```python
from build123d import *

# Parameters (mm, degrees)
CUT_EXTRUDE_1_DEPTH      = 205.5
CUT_EXTRUDE_1_DEPTH_BACK = 205.5
SKETCH_2_R               = 40
SKETCH_3_OUTSIDE_W       = 124.974
SKETCH_3_OUTSIDE_H       = 124.974
SKETCH_3_OUTSIDE_R       = 17.5
CUT_EXTRUDE_2_DEPTH      = 18
SKETCH_4_OUTSIDE_W       = 124.974
SKETCH_4_OUTSIDE_H       = 124.974
SKETCH_4_OUTSIDE_R       = 12.5
CUT_EXTRUDE_3_DEPTH      = 26
SKETCH_5_OUTSIDE_W       = 124.974
SKETCH_5_OUTSIDE_H       = 124.974
SKETCH_5_OUTSIDE_R       = 17.5
CUT_EXTRUDE_4_DEPTH      = 30
CUT_EXTRUDE_5_DEPTH      = 4
SKETCH_7_R               = 17.5
EXTRUDE_1_DEPTH          = 51
SKETCH_9_OUTSIDE_W       = 135.09
SKETCH_9_OUTSIDE_H       = 135.09
SKETCH_9_OUTSIDE_R       = 12
CUT_EXTRUDE_7_DEPTH      = 26
MOVE_FACE_1_BY           = 8


with BuildPart() as part:
    # 草图1 → 旋转1 (revolve)
    with BuildSketch(Plane.XY, mode=Mode.PRIVATE) as revolve_1_sk:
        Polygon((-205.5, 0), (-205.5, 19), (-204.5, 20), (204.5, 20), (205.5, 19), (205.5, 0), align=None)
    revolve(revolve_1_sk.sketch.rotate(Axis((205.5, 0, 0), (-1, 0, 0)), 270), axis=Axis((205.5, 0, 0), (-1, 0, 0)))

    # 草图2 → 切除-拉伸1 (cut, two sides: drawn at the far end of the back side and taken through both)
    with BuildSketch(Plane(origin=(0, 0, 0), x_dir=(0, 0, -1), z_dir=(1, 0, 0)).offset(-CUT_EXTRUDE_1_DEPTH_BACK)):
        Circle(SKETCH_2_R)
        with BuildLine():
            ThreePointArc((-19.926297295, 1.715423015), (-14.142135624, -14.142135624), (1.715423015, -19.926297295))
            ThreePointArc((1.715423015, -19.926297295), (3.302788339, -18.731043462), (5.203224708, -19.311303753))
            ThreePointArc((5.203224708, -19.311303753), (14.142135624, -14.142135624), (19.311303753, -5.203224708))
            ThreePointArc((19.311303753, -5.203224708), (18.731043462, -3.302788339), (19.926297295, -1.715423015))
            ThreePointArc((19.926297295, -1.715423015), (14.142135624, 14.142135624), (-1.715423015, 19.926297295))
            ThreePointArc((-1.715423015, 19.926297295), (-3.302788339, 18.731043462), (-5.203224708, 19.311303753))
            ThreePointArc((-5.203224708, 19.311303753), (-14.142135624, 14.142135624), (-19.311303753, 5.203224708))
            ThreePointArc((-19.311303753, 5.203224708), (-18.731043462, 3.302788339), (-19.926297295, 1.715423015))
        make_face(mode=Mode.SUBTRACT)
    extrude(amount=CUT_EXTRUDE_1_DEPTH + CUT_EXTRUDE_1_DEPTH_BACK, mode=Mode.SUBTRACT)

    # 草图3 outside → 切除-拉伸2 (cut)
    with BuildSketch(Plane.ZY.offset(205.5)):
        Rectangle(SKETCH_3_OUTSIDE_W, SKETCH_3_OUTSIDE_H)
        Circle(SKETCH_3_OUTSIDE_R, mode=Mode.SUBTRACT)
    extrude(amount=-CUT_EXTRUDE_2_DEPTH, mode=Mode.SUBTRACT)

    # 草图4 outside → 切除-拉伸3 (cut)
    with BuildSketch(Plane(origin=(205.5, 0, 0), x_dir=(0, 0, -1), z_dir=(1, 0, 0))):
        Rectangle(SKETCH_4_OUTSIDE_W, SKETCH_4_OUTSIDE_H)
        Circle(SKETCH_4_OUTSIDE_R, mode=Mode.SUBTRACT)
    extrude(amount=-CUT_EXTRUDE_3_DEPTH, mode=Mode.SUBTRACT)

    # 草图5 outside → 切除-拉伸4 (cut)
    with BuildSketch(Plane(origin=(179.5, 0, 0), x_dir=(0, 0, -1), z_dir=(1, 0, 0))):
        Rectangle(SKETCH_5_OUTSIDE_W, SKETCH_5_OUTSIDE_H)
        with Locations(Location((0, 0, 0), (0, 0, 180))):
            Circle(SKETCH_5_OUTSIDE_R, mode=Mode.SUBTRACT)
    extrude(amount=-CUT_EXTRUDE_4_DEPTH, mode=Mode.SUBTRACT)

    # 草图6 → 切除-拉伸5 (cut)
    with BuildSketch(Plane(origin=(0, 12.5, 0), x_dir=(1, 0, 0), z_dir=(0, 1, 0))):
        with BuildLine():
            Line((200.5, -4), (185.5, -4))
            ThreePointArc((185.5, -4), (181.5, 0), (185.5, 4))
            Line((185.5, 4), (200.5, 4))
            ThreePointArc((200.5, 4), (204.5, 0), (200.5, -4))
        make_face()
    cut_extrude_5 = extrude(amount=-CUT_EXTRUDE_5_DEPTH, mode=Mode.SUBTRACT)

    # 草图7 → 凸台-拉伸1 (add)
    with BuildSketch(Plane.ZY.offset(205.5)):
        Circle(SKETCH_7_R)
    extrude(amount=EXTRUDE_1_DEPTH)

    # 草图9 outside → 切除-拉伸7 (cut)
    with BuildSketch(Plane.ZY.offset(256.5)):
        Rectangle(SKETCH_9_OUTSIDE_W, SKETCH_9_OUTSIDE_H)
        Circle(SKETCH_9_OUTSIDE_R, mode=Mode.SUBTRACT)
    extrude(amount=-CUT_EXTRUDE_7_DEPTH, mode=Mode.SUBTRACT)

    # 镜向1: 切除-拉伸5 across plane
    add(cut_extrude_5.mirror(Plane.ZY.offset(25.5)), mode=Mode.SUBTRACT)

    # Move Face 1: a face moved outward by 8.0
    extrude(part.faces().sort_by_distance((-187.5, -16, -10))[0], amount=MOVE_FACE_1_BY, dir=(-1, 0, 0))


solid = part.part
```
Work out the finished part from the listing and answer in its coordinate system (mm). A direction names the side the tool comes from. Give positions to 0.01 mm unless a question says otherwise; leave off trailing zeros. Write each loop counter-clockwise with the first axis right and the second up, starting at its lowest first coordinate (ties: lowest second). Pieces come first, ordered by that corner, then holes. Notation, with made-up numbers: (3, 83.25) -> (18, 83.25) arc R9 ccw to (18, 89.25) -> close; hole circle Ø10 at (-35.5, 43.25). An arc over 180 degrees is marked (long way). Write each question's results on one line, items separated by ' | '.
1. A tool of negligible diameter and unlimited length cuts with its end or side. For faces 5 (the flat face through (-256.5, 0, 0)), 6 (the flat face through (193, 8.5, 0)), 7 (the cylindrical face through (-243.682, -11.715, -2.601)), 8 (the cylindrical face through (192.68, -11.09, -5.77)), from which of +Z, -Z, +X, -X, +Y, -Y can it reach the whole face along a straight path? Write none if from no direction.
Data:
face 5: +Z, -Z, -X, +Y, -Y | face 6: +Y | face 7: -X | face 8: +X
2. Straight lines are drawn through the part: L1, parallel to Y at x = -178.5, z = 5.5; L2, parallel to X at y = 11.5, z = -12; L3, parallel to Y at x = -94, z = 7 (3 decimals). For each, find the intervals that lie inside material, in ascending order.
Data:
L1: -19.23 to 19.23 | L2: -230.5 to 179.5 | L3: -18.735 to 18.735
3. Each of these flat-tipped pins is pushed along its axis until it touches: pin 1 Ø3 at (x, z) = (-144.5, -12.5) entering from +Y; pin 2 Ø1.4 at (x, y) = (-246, 10.5) entering from -Z; pin 3 Ø4 at (x, y) = (114, -16) entering from +Z. Where does it stop, or does it pass through?
Data:
pin 1: y = 16.7 | pin 2: z = -6.93 | pin 3: z = 14.28
4. Determine the mould class of faces 1 (the cylindrical face through (-20.59, -13.97, 14.31)), 2 (the flat face through (-244, 8.5, 0)), 3 (the flat face through (205.5, 0, 0)), 4 (the flat face through (-195.5, -18, 0)) for opening direction X: +X half, -X half, draft (parallel to the pull), parting line (faces both ways), or undercut.
Data:
face 1: draft | face 2: undercut | face 3: +X half | face 4: -X half
5. Find section A-A on x = 42. Determine the outline of the cut face in (y, z), and give its area (3 significant figures).
Data:
outline: (-19.93, -1.72) arc R2.19 cw to (-19.31, -5.2) arc R20 ccw to (-5.2, -19.31) arc R2.19 cw to (-1.72, -19.93) arc R20 ccw to (19.93, 1.72) arc R2.19 cw to (19.31, 5.2) arc R20 ccw to (5.2, 19.31) arc R2.19 cw to (1.72, 19.93) arc R20 ccw to start | area: 1,250 mm^2
